from build123d import *

# Parameters (mm, degrees)
SKETCH_1_W               = 80
SKETCH_1_H               = 80
EXTRUDE_1_DEPTH          = 24
FILLET_1_R               = 10
SKETCH_2_R               = 4
CUT_EXTRUDE_1_DEPTH      = 62.449165983
MIRROR_2_COPY_1_SKETCH_R = 4
MIRROR_2_COPY_1_DEPTH    = 62.449165983
SKETCH_3_R               = 30
EXTRUDE_2_DEPTH          = 2.5
SKETCH_4_R               = 10
CUT_EXTRUDE_2_DEPTH      = 49.5
CUT_EXTRUDE_3_DEPTH      = 2.5


with BuildPart() as part:
    # 草图1 → 凸台-拉伸1 (new body)
    with BuildSketch(Plane.XY):
        Rectangle(SKETCH_1_W, SKETCH_1_H)
    extrude(amount=EXTRUDE_1_DEPTH)

    # 圆角1
    fillet_1_edges = [part.edges().sort_by_distance(p)[0] for p in [
        (40, -40, 12),
        (-40, -40, 12),
        (-40, 40, 12),
        (40, 40, 12),
    ]]
    fillet(fillet_1_edges, radius=FILLET_1_R)

    # 草图2 → 切除-拉伸1 (cut, symmetric)
    with BuildSketch(Plane.XY.offset(24)):
        with Locations((-30.5, 30.5)):
            Circle(SKETCH_2_R)
    cut_extrude_1 = extrude(amount=CUT_EXTRUDE_1_DEPTH, both=True, mode=Mode.SUBTRACT)

    # 镜向1: 切除-拉伸1 across plane
    add(cut_extrude_1.mirror(Plane.ZX), mode=Mode.SUBTRACT)

    # 镜向2: 切除-拉伸1 across plane
    add(cut_extrude_1.mirror(Plane(origin=(0, 0, 0), x_dir=(0, 0, 1), z_dir=(1, 0, 0))), mode=Mode.SUBTRACT)

    # 镜向2 copy 1 sketch → 镜向2 copy 1 (cut, symmetric)
    with BuildSketch(Plane(origin=(0, 0, 24), x_dir=(-1, 0, 0), z_dir=(0, 0, 1))):
        with Locations((-30.5, 30.5)):
            Circle(MIRROR_2_COPY_1_SKETCH_R)
    extrude(amount=MIRROR_2_COPY_1_DEPTH, both=True, mode=Mode.SUBTRACT)

    # 草图3 → 凸台-拉伸2 (add)
    with BuildSketch(Plane.XY.offset(24)):
        with Locations(Location((0, 0, 0), (0, 0, 180))):
            Circle(SKETCH_3_R)
    extrude(amount=EXTRUDE_2_DEPTH)

    # 草图4 → 切除-拉伸2 (cut)
    with BuildSketch(Plane.XY.offset(26.5)):
        Circle(SKETCH_4_R)
    extrude(amount=-CUT_EXTRUDE_2_DEPTH, mode=Mode.SUBTRACT)

    # 草图5 → 切除-拉伸3 (cut)
    with BuildSketch(Plane(origin=(0, 0, 0), x_dir=(-1, 0, 0), z_dir=(0, 0, -1))):
        with BuildLine():
            Line((-23.263481458, -25.438517127), (23.263481458, -25.438517127))
            ThreePointArc((23.263481458, -25.438517127), (24.677695021, -24.852730689), (25.263481458, -23.438517127))
            Line((25.263481458, -23.438517127), (25.263481458, 23.438517127))
            ThreePointArc((25.263481458, 23.438517127), (24.677695021, 24.852730689), (23.263481458, 25.438517127))
            Line((23.263481458, 25.438517127), (-23.263481458, 25.438517127))
            ThreePointArc((-23.263481458, 25.438517127), (-24.677695021, 24.852730689), (-25.263481458, 23.438517127))
            Line((-25.263481458, 23.438517127), (-25.263481458, -23.438517127))
            ThreePointArc((-25.263481458, -23.438517127), (-24.677695021, -24.852730689), (-23.263481458, -25.438517127))
        make_face()
    extrude(amount=-CUT_EXTRUDE_3_DEPTH, mode=Mode.SUBTRACT)


solid = part.part
For this review, take the finished solid that the model builds, in its own axes (mm). A direction names the side the tool comes from. Round coordinates to 2 decimals unless told otherwise and drop trailing zeros. Write each loop counter-clockwise with the first axis right and the second up, starting at its lowest first coordinate (ties: lowest second). Pieces come first, ordered by that corner, then holes. Notation, with made-up numbers: (65, 1.25) -> (121, 1.25) arc R15 ccw to (121, 28.25) -> close; hole circle Ø2 at (34.5, 37.5). An arc over 180 degrees is marked (long way). Use CSV: the item, a comma, the result in double quotes.
(1) Consider section A-A, the plane x = 0. Give the boundary of the cut face in (y, z).
Computed values:
outline,"(-40, 0) -> (-25.44, 0) -> (-25.44, 2.5) -> (-10, 2.5) -> (-10, 26.5) -> (-30, 26.5) -> (-30, 24) -> (-40, 24) -> close; (10, 2.5) -> (25.44, 2.5) -> (25.44, 0) -> (40, 0) -> (40, 24) -> (30, 24) -> (30, 26.5) -> (10, 26.5) -> close"
(2) Consider section B-B, the plane y = 0. Give the boundary of the cut face in (x, z).
Computed values:
outline,"(-40, 0) -> (-25.26, 0) -> (-25.26, 2.5) -> (-10, 2.5) -> (-10, 26.5) -> (-30, 26.5) -> (-30, 24) -> (-40, 24) -> close; (10, 2.5) -> (25.26, 2.5) -> (25.26, 0) -> (40, 0) -> (40, 24) -> (30, 24) -> (30, 26.5) -> (10, 26.5) -> close"
(3) Consider section D-D, the plane y = 16. Give the boundary of the cut face in (x, z).
Computed values:
outline,"(-40, 0) -> (-25.26, 0) -> (-25.26, 2.5) -> (25.26, 2.5) -> (25.26, 0) -> (40, 0) -> (40, 24) -> (25.38, 24) -> (25.38, 26.5) -> (-25.38, 26.5) -> (-25.38, 24) -> (-40, 24) -> close"
(4) To check wall thickness, follow L1, parallel to Y at x = 30.5, z = 6.5; L2, parallel to Y at x = -12, z = 2.25; L3, parallel to Z at x = 35.5, y = -24. State the ranges of each line that lie inside material, in increasing order. Write a range as [from, to].
Computed values:
L1,"[-39.99, -34.5], [-26.5, 26.5], [34.5, 39.99]"
L2,"[-40, -25.44], [25.44, 40]"
L3,"[0, 24]"
(5) Draft analysis for pull direction Y (two halves, no side actions). For faces 1 (the face through (40, 0, 12)), 2 (the face through (-24.66, -24.87, 1.23)), 3 (the face through (-37.15, 36.99, 12.17)), state which applies: +Y half, -Y half, draft (parallel to the pull), parting line (faces both ways), or undercut.
Computed values:
face 1,"draft"
face 2,"undercut"
face 3,"+Y half"
(6) For faces 4 (the face through (31.021, -34.466, 12.168)), 5 (the face through (-16.128, -25.296, 25.232)), 6 (the face through (24.69, -24.84, 1.23)), list the 3-axis set-ups (+Z, -Z, +X, -X, +Y, -Y) from which the entire face can be reached by the end or side of a thin tool; tool diameter is ignored.
Computed values:
face 4,"+Z, -Z"
face 5,"+Z"
face 6,"-Z"
(7) Consider section C-C, the plane z = 11.25. Give the boundary of the cut face in (x, y), plus the area to 3 significant figures.
Computed values:
outline,"(-40, -30) arc R10 ccw to (-30, -40) -> (30, -40) arc R10 ccw to (40, -30) -> (40, 30) arc R10 ccw to (30, 40) -> (-30, 40) arc R10 ccw to (-40, 30) -> close; hole circle Ø8 at (-30.5, -30.5); hole circle Ø8 at (-30.5, 30.5); hole circle Ø20 at (0, 0); hole circle Ø8 at (30.5, -30.5); hole circle Ø8 at (30.5, 30.5)"
area,"5,800 mm²"
(8) Clearance check with flat-ended pins moving along their axes: P1, Ø10.5, axis at x = 30.5, y = 30.5, coming from the +Z side; P2, Ø6.5, axis at x = -30.5, y = -30.5, coming from the -Z side; P3, Ø1, axis at x = -6.5, y = 9.5, coming from the -Z side. State where each tip first meets the part, or that it passes through.
Computed values:
P1,"z = 24"
P2,"through"
P3,"z = 2.5"
